```python
from build123d import *

# Parameters (mm, degrees)
BRACKET_PROFILE_SKETCH_R   = 30
BRACKET_PROFILE_SKETCH_R_2 = 25
BRACKET_PROFILE_SKETCH_R_3 = 40
BRACKET_PLATE_50MM_DEPTH   = 25


with BuildPart() as part:
    # Bracket Profile Sketch → Bracket Plate 50mm (new, symmetric)
    with BuildSketch(Plane.XY):
        with BuildLine():
            Line((-393.337365548, 211.308411215), (-393.337365548, -248.691588785))
            ThreePointArc((-393.337365548, -248.691588785), (-387.479501171, -262.833724409), (-373.337365548, -268.691588785))
            Line((-373.337365548, -268.691588785), (-213.337365548, -268.691588785))
            ThreePointArc((-213.337365548, -268.691588785), (-199.195229924, -262.833724409), (-193.337365548, -248.691588785))
            Line((-193.337365548, -248.691588785), (-193.337365548, -213.676012461))
            ThreePointArc((-193.337365548, -213.676012461), (-181.621636795, -185.391741214), (-153.337365548, -173.676012461))
            Line((-153.337365548, -173.676012461), (316.662634452, -173.676012461))
            ThreePointArc((316.662634452, -173.676012461), (344.9469057, -185.391741214), (356.662634452, -213.676012461))
            Line((356.662634452, -213.676012461), (356.662634452, -248.691588785))
            ThreePointArc((356.662634452, -248.691588785), (362.520498829, -262.833724409), (376.662634452, -268.691588785))
            Line((376.662634452, -268.691588785), (536.662634452, -268.691588785))
            ThreePointArc((536.662634452, -268.691588785), (550.804770076, -262.833724409), (556.662634452, -248.691588785))
            Line((556.662634452, -248.691588785), (556.662634452, -88.691588785))
            ThreePointArc((556.662634452, -88.691588785), (550.804770076, -74.549453161), (536.662634452, -68.691588785))
            Line((536.662634452, -68.691588785), (336.307967431, -68.691588785))
            ThreePointArc((336.307967431, -68.691588785), (150.648831804, -20.2495556), (12.324990963, 112.725856698))
            ThreePointArc((12.324990963, 112.725856698), (5.044788813, 119.724562608), (-4.726744641, 122.274143302))
            Line((-4.726744641, 122.274143302), (-173.337365548, 122.274143302))
            ThreePointArc((-173.337365548, 122.274143302), (-187.479501171, 128.132007678), (-193.337365548, 142.274143302))
            Line((-193.337365548, 142.274143302), (-193.337365548, 211.308411215))
            ThreePointArc((-193.337365548, 211.308411215), (-199.195229924, 225.450546839), (-213.337365548, 231.308411215))
            Line((-213.337365548, 231.308411215), (-373.337365548, 231.308411215))
            ThreePointArc((-373.337365548, 231.308411215), (-387.479501171, 225.450546839), (-393.337365548, 211.308411215))
        make_face()
        with Locations((-293.337365548, 131.308411215)):
            Circle(BRACKET_PROFILE_SKETCH_R, mode=Mode.SUBTRACT)
        with Locations((-293.337365548, -168.691588785)):
            Circle(BRACKET_PROFILE_SKETCH_R, mode=Mode.SUBTRACT)
        with Locations((-43.337365548, -18.691588785)):
            Circle(BRACKET_PROFILE_SKETCH_R_2, mode=Mode.SUBTRACT)
        with Locations((456.662634452, -168.691588785)):
            Circle(BRACKET_PROFILE_SKETCH_R_3, mode=Mode.SUBTRACT)
    extrude(amount=BRACKET_PLATE_50MM_DEPTH, both=True)


solid = part.part
```
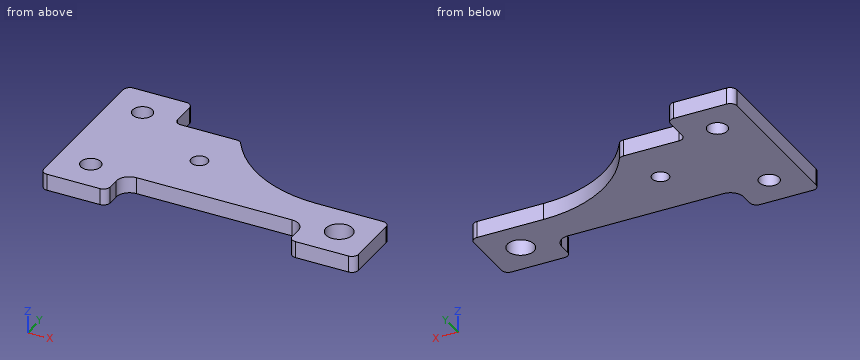
Build history of the part. All positions in model axes, mm. Coordinates: 2 decimals unless noted, no trailing zeros. Order: outer loops, then holes, each group sorted by start corner. A loop starts at its lowest first (then second) coordinate and runs counter-clockwise, first axis right, second up. Notation, with made-up numbers: M -36.5,47 L -28.5,47 A13 cw -28.5,69 Z; hole C 79.25,22.25 d2. An arc over 180 degrees is marked long. One line per question, with ' | ' between items. Start each with the question number.
1. Cut at B-B (y = -151.5). Write the cut outline in (x, z), plus the area to 3 significant figures.
2. Cut at C-C (x = 405). Write the cut outline in (y, z), plus the area to 3 significant figures.
3. Wall check: line 1 along Y through (x, z) = (-274, -4); line 2 along X through (y, z) = (-240, -12); line 3 along X through (y, z) = (-183.5, 10). Give the ranges that are in metal, low to high. Write a range as [from, to].
4. Cut at D-D (y = 18). Write the cut outline in (x, z).
5. Flat gauge pins, fed straight in: P1, Ø3, axis at x = 141, z = 0.5, coming from the +Y side; P2, Ø2, axis at x = 183.5, z = 10.5, coming from the -Y side. Where does each tip first touch, or does it go through?
6. Cut at A-A (z = -6). Write the cut outline in (x, y) (3 decimals).
The answers:
1) outline: M -393.34,-25 L -317.92,-25 L -317.92,25 L -393.34,25 Z; M -268.75,-25 L 420.55,-25 L 420.55,25 L -268.75,25 Z; M 492.78,-25 L 556.66,-25 L 556.66,25 L 492.78,25 Z | area: 41,400 mm2
2) outline: M -268.69,-25 L -68.69,-25 L -68.69,25 L -268.69,25 Z | area: 10,000 mm2
3) line 1: y = [-268.69, -191.63], [-145.76, 108.37], [154.24, 231.31] | line 2: x = [-393.34, -193.34], [356.66, 556.66] | line 3: x = [-393.34, -319.43], [-267.25, -179.59], [342.92, 419.5], [493.82, 556.66]
4) outline: M -393.34,-25 L 94.71,-25 L 94.71,25 L -393.34,25 Z
5) P1: stops at y = -13.76 | P2: stops at y = -173.68
6) outline: M -393.337,-248.692 A20 ccw -373.337,-268.692 L -213.337,-268.692 A20 ccw -193.337,-248.692 L -193.337,-213.676 A40 cw -153.337,-173.676 L 316.663,-173.676 A40 cw 356.663,-213.676 L 356.663,-248.692 A20 ccw 376.663,-268.692 L 536.663,-268.692 A20 ccw 556.663,-248.692 L 556.663,-88.692 A20 ccw 536.663,-68.692 L 336.308,-68.692 A380 cw 12.325,112.726 A20 ccw -4.727,122.274 L -173.337,122.274 A20 cw -193.337,142.274 L -193.337,211.308 A20 ccw -213.337,231.308 L -373.337,231.308 A20 ccw -393.337,211.308 Z; hole C -293.337,-168.692 d60; hole C -293.337,131.308 d60; hole C -43.337,-18.692 d50; hole C 456.663,-168.692 d80
